Design review of the part built by this model. Coordinates are the model's own, in mm. A direction names the side the tool comes from. Coordinates: 2 decimals unless noted, no trailing zeros. Loops run counter-clockwise (first coordinate to the right, second up) from the corner with the lowest first, then second, coordinate; pieces in that order, holes last. Notation, with made-up numbers: (79.25, -33) -> (93.25, -33) arc R8 cw to (93.25, -26) -> close; hole circle Ø11 at (57.25, 51.25). An arc over 180 degrees is marked (long way). Use a Markdown table: item, result. Add a question column.
Q1. Take a section at B-B on z = 1.45. Write out the cut boundary in (x, y).
Q2. For probe 1 along X at (y, z) = (-57, 2); probe 2 along X at (y, z) = (-51, 0.2); probe 3 along X at (y, z) = (-97.5, 2.4), list the stretches that pass through material, from the lowest coordinate up.
Q3. Take a section at D-D on x = 88. Write out the cut boundary in (y, z), plus the area to 3 significant figures.
Q4. Take a section at A-A on y = -38. Write out the cut boundary in (x, z).
Q5. Take a section at C-C on y = -118.5. Write out the cut boundary in (x, z), plus the area to 3 significant figures.
Q6. For faces 1 (the face through (86, -22, 1)), 2 (the face through (19, -150, 1)), list the 3-axis set-ups (+Z, -Z, +X, -X, +Y, -Y) from which the entire face can be reached by the end or side of a thin tool; tool diameter is ignored.
from build123d import *

# Parameters (mm, degrees)
BOSS_EXTRUDE1_DEPTH = 3


with BuildPart() as part:
    # Sketch1 → Boss-Extrude1 (new body)
    with BuildSketch(Plane.XY):
        with BuildLine():
            Line((0, -5), (0, -145))
            ThreePointArc((0, -145), (1.464466094, -148.535533906), (5, -150))
            Line((5, -150), (33.638458538, -150))
            ThreePointArc((33.638458538, -150), (34.952164103, -149.824331839), (36.173559171, -149.309671076))
            Line((36.173559171, -149.309671076), (117.535100633, -101.449940804))
            ThreePointArc((117.535100633, -101.449940804), (119.340247871, -99.622657373), (120, -97.140269728))
            Line((120, -97.140269728), (120, -5))
            ThreePointArc((120, -5), (118.535533906, -1.464466094), (115, 0))
            Line((115, 0), (91, 0))
            ThreePointArc((91, 0), (87.464466094, -1.464466094), (86, -5))
            Line((86, -5), (86, -40))
            ThreePointArc((86, -40), (60, -66), (34, -40))
            Line((34, -40), (34, -5))
            ThreePointArc((34, -5), (32.535533906, -1.464466094), (29, 0))
            Line((29, 0), (5, 0))
            ThreePointArc((5, 0), (1.464466094, -1.464466094), (0, -5))
        make_face()
    extrude(amount=BOSS_EXTRUDE1_DEPTH)


solid = part.part
Answer list:
| question | item | result |
|---|---|---|
| 1 | outline | (0, -145) arc R5 ccw to (5, -150) -> (33.64, -150) arc R5 ccw to (36.17, -149.31) -> (117.54, -101.45) arc R5 ccw to (120, -97.14) -> (120, -5) arc R5 ccw to (115, 0) -> (91, 0) arc R5 ccw to (86, -5) -> (86, -40) arc R26 cw to (34, -40) -> (34, -5) arc R5 ccw to (29, 0) -> (5, 0) arc R5 ccw to (0, -5) -> close |
| 2 | probe 1 | 0 to 40.33, 79.67 to 120 |
| 2 | probe 2 | 0 to 36.44, 83.56 to 120 |
| 2 | probe 3 | 0 to 119.99 |
| 3 | outline | (-118.82, 0) -> (-1, 0) -> (-1, 3) -> (-118.82, 3) -> close |
| 3 | area | 353 mm² |
| 4 | outline | (0, 0) -> (34, 0) -> (34, 3) -> (0, 3) -> close; (86, 0) -> (120, 0) -> (120, 3) -> (86, 3) -> close |
| 5 | outline | (0, 0) -> (88.55, 0) -> (88.55, 3) -> (0, 3) -> close |
| 5 | area | 266 mm² |
| 6 | face 1 | +Z, -Z, +Y |
| 6 | face 2 | +Z, -Z, +X, -X, -Y |
